```python
from build123d import *

# Parameters (mm, degrees)
SKETCH1_W              = 170
SKETCH1_H              = 170
EXTRUDE1_DEPTH         = 12
M16X2_0_TAPPED_HOLE1_D = 14
CHAMFER1_SIZE          = 65


with BuildPart() as part:
    # Sketch1 → Extrude1 (new body)
    with BuildSketch(Plane.XY):
        with Locations((85, 85)):
            Rectangle(SKETCH1_W, SKETCH1_H)
    extrude(amount=-EXTRUDE1_DEPTH)

    # M16x2.0 Tapped Hole1 (through all)
    with Locations(Plane.XY):
        with Locations((20, 20)):
            Hole(M16X2_0_TAPPED_HOLE1_D / 2)

    # Chamfer1
    chamfer1_edges = [part.edges().sort_by_distance(p)[0] for p in [
        (170, 170, -6),
    ]]
    chamfer(chamfer1_edges, length=CHAMFER1_SIZE)


solid = part.part
```
The listing builds one solid part. Answer for the finished solid, in the listing's coordinates (mm). Round coordinates to 2 decimals unless told otherwise and drop trailing zeros. Loops run counter-clockwise (first coordinate to the right, second up) from the corner with the lowest first, then second, coordinate; pieces in that order, holes last.
1) A cutting plane is placed at D-D on x = 116. Determine the outline of the cut face in (y, z).
Outcome:
outline: (0, -12) - (159, -12) - (159, 0) - (0, 0) - close
2) For a pull along X with two mould halves and no side action, classify faces 1 (the face through (138, 137, -6)), 2 (the face through (21.517, 13.166, -6.084)), 3 (the face through (84, 86, 0)), 4 (the face through (0, 84, -6)) as released by +X, released by -X, zero draft, split by the parting line, or undercut.
Outcome:
face 1: released by +X
face 2: undercut
face 3: zero draft
face 4: released by -X
3) A cutting plane is placed at C-C on y = 22. Determine the outline of the cut face in (x, z), plus the area to 3 significant figures.
Outcome:
outline: (0, -12) - (13.29, -12) - (13.29, 0) - (0, 0) - close; (26.71, -12) - (170, -12) - (170, 0) - (26.71, 0) - close
area: 1,880 mm2
4) A cutting plane is placed at B-B on z = -8.5. Determine the outline of the cut face in (x, y).
Outcome:
outline: (0, 0) - (170, 0) - (170, 105) - (105, 170) - (0, 170) - close; hole circle Ø14 at (20, 20)
5) Consider line 1 (Y direction, x = 20, z = -7.5); line 2 (Y direction, x = 139, z = -5.25); line 3 (Y direction, x = 123.5, z = -7). Determine where each line is inside the solid, lowest interval first.
Outcome:
line 1: y = 0 to 13, 27 to 170
line 2: y = 0 to 136
line 3: y = 0 to 151.5
6) A cutting plane is placed at A-A on x = 20. Determine the outline of the cut face in (y, z), plus the area to 3 significant figures.
Outcome:
outline: (0, -12) - (13, -12) - (13, 0) - (0, 0) - close; (27, -12) - (170, -12) - (170, 0) - (27, 0) - close
area: 1,870 mm2
7) Given P1, Ø1.5, axis at x = 133, z = -2, coming from the +Y side, flat-ended and moving along its own axis, determine where the tip first touches the part or whether it passes through.
Outcome:
P1: stops at y = 142.75
